The model under review builds one solid part; all positions refer to its coordinate system, in mm. Face numbers are marked on the shaded views. Coordinates: 2 decimals unless noted, no trailing zeros. Write each loop counter-clockwise with the first axis right and the second up, starting at its lowest first coordinate (ties: lowest second). Pieces come first, ordered by that corner, then holes.
1) Add section A-A, the plane x = 0. State the section outline as (y, z) points.
2) Add section D-D, the plane x = 9.25. State the section outline as (y, z) points, then the cut area to 3 significant figures.
3) Add section C-C, the plane z = -4.25. State the section outline as (x, y) points, then the cut area to 3 significant figures.
4) Mouldability with a two-part tool opening along X and no side actions: class the marked faces 1, 2, 3 and 4 as released by +X, released by -X, zero draft, split by the parting line, or undercut.
5) For P1, Ø8, axis at x = -4, z = 4, coming from the -Y side; P2, Ø1, axis at y = 105, z = 4.5, coming from the +X side; P3, Ø1.5, axis at y = 93, z = -2.5, coming from the +X side; P4, Ø4, axis at y = 68, z = 6.5, coming from the -X side, all flat-tipped, find the tip position at first contact; note any pin that passes through.
6) For line 1 (Z direction, x = 0, y = 34); line 2 (X direction, y = 46.5, z = 0); line 3 (Z direction, x = -1.25, y = 23.5), list the stretches that pass through material, from the lowest coordinate up.
7) Add section B-B, the plane y = 70. State the section outline as (x, z) points.
from build123d import *

# Parameters (mm, degrees)
BOSS_EXTRUDE1_DEPTH = 63.5
SKETCH2_R           = 2.667
CUT_EXTRUDE1_DEPTH  = 127
SCALE1_SCALE        = 2


with BuildPart() as part:
    # Sketch1 → Boss-Extrude1 (new body)
    with BuildSketch(Plane(origin=(0, 0, 0), x_dir=(1, 0, 0), z_dir=(0, 1, 0))):
        Polygon((2.932939367, -5.08), (5.865878735, 0), (2.932939367, 5.08), (-2.932939367, 5.08), (-5.865878735, 0), (-2.932939367, -5.08), align=None)
    extrude(amount=BOSS_EXTRUDE1_DEPTH)

    # Sketch2 → Cut-Extrude1 (cut)
    with BuildSketch(Plane(origin=(0, 0, 0), x_dir=(1, 0, 0), z_dir=(0, 1, 0))):
        with Locations(Location((0, 0, 0), (0, 0, 270))):
            Circle(SKETCH2_R)
    extrude(amount=CUT_EXTRUDE1_DEPTH, mode=Mode.SUBTRACT)


with BuildPart() as part_1:
    # Scale1: scaled about (0, 0, 0)
    add(part.part.scale(SCALE1_SCALE))


solid = part_1.part
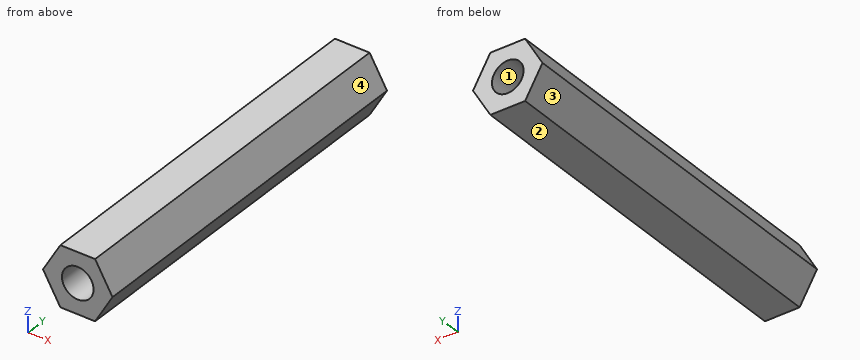
Geometry results:
1. outline: (0, -10.16) - (127, -10.16) - (127, -5.33) - (0, -5.33) - close; (0, 5.33) - (127, 5.33) - (127, 10.16) - (0, 10.16) - close
2. outline: (0, -4.3) - (127, -4.3) - (127, 4.3) - (0, 4.3) - close
2. area: 1,090 mm2
3. outline: (-9.28, 0) - (-3.22, 0) - (-3.22, 127) - (-9.28, 127) - close; (3.22, 0) - (9.28, 0) - (9.28, 127) - (3.22, 127) - close
3. area: 1,540 mm2
4. face 1: undercut
4. face 2: zero draft
4. face 3: released by -X
4. face 4: released by +X
5. P1: stops at y = 0
5. P2: stops at x = 9.42
5. P3: stops at x = 10.72
5. P4: stops at x = -9.13
6. line 1: z = -10.16 to -5.33, 5.33 to 10.16
6. line 2: x = -11.73 to -5.33, 5.33 to 11.73
6. line 3: z = -10.16 to -5.19, 5.19 to 10.16
7. outline: (-11.73, 0) - (-5.87, -10.16) - (5.87, -10.16) - (11.73, 0) - (5.87, 10.16) - (-5.87, 10.16) - close; hole circle Ø10.67 at (0, 0)
